from build123d import *

# Parameters (mm, degrees)
BASE_PLATE_DEPTH          = 150
WEB_RIB_DEPTH             = 3
TALL_BOSS_PROFILE_R       = 17.5
TALL_BOSS_35_DEPTH        = 90
TALL_BOSS_BORE_PROFILE_R  = 6
TALL_BOSS_BORE_12_DEPTH   = 204.155113152
SHORT_BOSS_PROFILE_R      = 20
SHORT_BOSS_40_DEPTH       = 30
SHORT_BOSS_BORE_PROFILE_R = 7
SHORT_BOSS_BORE_14_DEPTH  = 179.538511252
SIDE_LUG_DEPTH            = 20


with BuildPart() as part:
    # Base Plate Profile → Base Plate (new body)
    with BuildSketch(Plane(origin=(0, 0, 0), x_dir=(0, 0, -1), z_dir=(1, 0, 0))):
        Polygon((0, 0), (0, 12), (76, 12), (76, 0), (52, 0), (52, -12), (24, -12), (24, 0), align=None)
    extrude(amount=BASE_PLATE_DEPTH)

    # Web Rib Profile → Web Rib (add, symmetric)
    with BuildSketch(Plane.XY.offset(-38)):
        Polygon((75, 12), (105, 12), (105, 102), (45, 42), (45, 12), align=None)
    extrude(amount=WEB_RIB_DEPTH, both=True)

    # Tall Boss Profile → Tall Boss Ø35 (add)
    with BuildSketch(Plane(origin=(0, 12, 0), x_dir=(1, 0, 0), z_dir=(0, 1, 0))):
        with Locations(Location((120, 38, 0), (0, 0, 170.129110394))):
            Circle(TALL_BOSS_PROFILE_R)
    extrude(amount=TALL_BOSS_35_DEPTH)

    # Tall Boss Bore Profile → Tall Boss Bore Ø12 (cut, through all)
    with BuildSketch(Plane(origin=(0, 102, 0), x_dir=(1, 0, 0), z_dir=(0, 1, 0))):
        with Locations(Location((120, 38, 0), (0, 0, 270))):
            Circle(TALL_BOSS_BORE_PROFILE_R)
    extrude(amount=-TALL_BOSS_BORE_12_DEPTH, mode=Mode.SUBTRACT)

    # Short Boss Profile → Short Boss Ø40 (add)
    with BuildSketch(Plane(origin=(0, 12, 0), x_dir=(1, 0, 0), z_dir=(0, 1, 0))):
        with Locations((30, 38)):
            Circle(SHORT_BOSS_PROFILE_R)
    extrude(amount=SHORT_BOSS_40_DEPTH)

    # Short Boss Bore Profile → Short Boss Bore Ø14 (cut, through all)
    with BuildSketch(Plane(origin=(0, 42, 0), x_dir=(1, 0, 0), z_dir=(0, 1, 0))):
        with Locations(Location((30, 38, 0), (0, 0, 270))):
            Circle(SHORT_BOSS_BORE_PROFILE_R)
    extrude(amount=-SHORT_BOSS_BORE_14_DEPTH, mode=Mode.SUBTRACT)

    # Side Lug Profile → Side Lug (add)
    with BuildSketch(Plane(origin=(150, 0, 0), x_dir=(0, 0, -1), z_dir=(1, 0, 0))):
        Polygon((38, 12), (28, 12), (28, 102), (48, 102), (48, 12), align=None)
    extrude(amount=-SIDE_LUG_DEPTH)


solid = part.part
The model under review builds one solid part; all positions refer to its coordinate system, in mm. A direction names the side the tool comes from. Round coordinates to 2 decimals unless told otherwise and drop trailing zeros. Loops run counter-clockwise (first coordinate to the right, second up) from the corner with the lowest first, then second, coordinate; pieces in that order, holes last. Notation, with made-up numbers: (-5, 52.25) - (16, 52.25) arc R4 cw to (16, 58.25) - close; hole circle Ø11 at (83.25, 26). An arc over 180 degrees is marked (long way). Use CSV: the item, a comma, the result in double quotes.
(1) Clearance check with flat-ended pins moving along their axes: P1, Ø2, axis at x = 105.5, y = 89.5, coming from the -Z side; P2, Ø8, axis at y = 81, z = -30.5, coming from the -X side; P3, Ø4.5, axis at x = 139.5, y = 47, coming from the -Z side. State where each tip first meets the part, or that it passes through.
Working result:
P1,"stops at z = -49.14"
P2,"stops at x = 102.85"
P3,"stops at z = -48"
(2) Take a section at D-D, the plane y = 89. Give the boundary of the cut face in (x, z), plus the area to 3 significant figures.
Working result:
outline,"(92, -41) - (102.76, -41) arc R17.5 ccw to (134.36, -48) - (150, -48) - (150, -28) - (134.36, -28) arc R17.5 ccw to (102.76, -35) - (92, -35) - close; hole circle Ø12 at (120, -38)"
area,"1,180 mm^2"
(3) Take a section at C-C, the plane y = 34.5. Give the boundary of the cut face in (x, z), plus the area to 3 significant figures.
Working result:
outline,"(49.77, -41) - (102.76, -41) arc R17.5 ccw to (134.36, -48) - (150, -48) - (150, -28) - (134.36, -28) arc R17.5 ccw to (102.76, -35) - (49.77, -35) arc R20 ccw (long way) to start; hole circle Ø14 at (30, -38); hole circle Ø12 at (120, -38)"
area,"2,540 mm^2"
(4) The part is to be moulded in two halves that separate along X. For faces 1 (the flat face through (80, 47, -35)), 2 (the cylindrical face through (27.319, 15.378, -31.534)), 3 (the flat face through (0, 3, -39)), 4 (the flat face through (127, 102, -38)), say which applies: pulls with the +X half, pulls with the -X half, needs draft (parallel to the pull), parting line crosses it, or undercut.
Working result:
face 1,"undercut"
face 2,"undercut"
face 3,"pulls with the -X half"
face 4,"needs draft"
(5) Take a section at A-A, the plane x = 120. Give the boundary of the cut face in (y, z).
Working result:
outline,"(-12, -52) - (0, -52) - (0, -76) - (12, -76) - (12, -55.5) - (102, -55.5) - (102, -44) - (-12, -44) - close; (-12, -32) - (102, -32) - (102, -20.5) - (12, -20.5) - (12, 0) - (0, 0) - (0, -24) - (-12, -24) - close"
(6) For line 1 (X direction, y = 24, z = -38); line 2 (X direction, y = 3.5, z = -38); line 3 (Y direction, x = 121, z = -14), list the stretches that pass through material, from the lowest coordinate up.
Working result:
line 1,"x = 10 to 23, 37 to 114, 126 to 150"
line 2,"x = 0 to 23, 37 to 114, 126 to 150"
line 3,"y = 0 to 12"
(7) Take a section at B-B, the plane z = -38. Give the boundary of the cut face in (x, y).
Working result:
outline,"(0, -12) - (23, -12) - (23, 42) - (10, 42) - (10, 12) - (0, 12) - close; (37, -12) - (114, -12) - (114, 102) - (102.5, 102) - (102.5, 99.5) - (45, 42) - (37, 42) - close; (126, -12) - (150, -12) - (150, 102) - (126, 102) - close"
(8) Machinability: for faces 5 (the flat face through (80, 47, -41)), 6 (the flat face through (142, 56, -28)), 7 (the flat face through (74, -6, -52)), 8 (the flat face through (142, 58, -48)), which of the approach directions +Z, -Z, +X, -X, +Y, -Y give a long, thin tool a straight path to every point of the face, cutting with its end or side? Answer none if there is none.
Working result:
face 5,"-Z, +Y"
face 6,"+Z, +X, +Y"
face 7,"-Z, +X, -X, -Y"
face 8,"-Z, +X, +Y"
